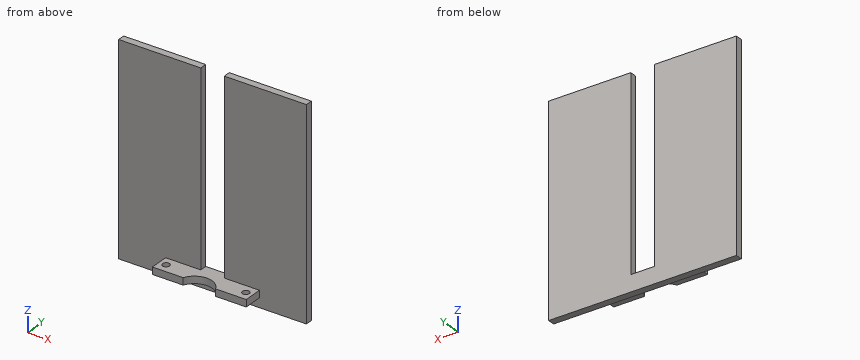
```python
from build123d import *

# Parameters (mm, degrees)
SKETCH2_R           = 1.5
BOSS_EXTRUDE1_DEPTH = 3
BOSS_EXTRUDE2_DEPTH = 3


with BuildPart() as part:
    # Sketch2 → Boss-Extrude1 (new body)
    with BuildSketch(Plane.XY):
        with BuildLine():
            Line((-20, 3), (-6.873863542, 3))
            ThreePointArc((-6.873863542, 3), (0, 7.5), (6.873863542, 3))
            Line((6.873863542, 3), (20, 3))
            Line((20, 3), (20, 11))
            Line((20, 11), (-20, 11))
            Line((-20, 11), (-20, 3))
        make_face()
        with Locations((-17, 7)):
            Circle(SKETCH2_R, mode=Mode.SUBTRACT)
        with Locations((17, 7)):
            Circle(SKETCH2_R, mode=Mode.SUBTRACT)
    extrude(amount=BOSS_EXTRUDE1_DEPTH)

    # Sketch3 → Boss-Extrude2 (add)
    with BuildSketch(Plane(origin=(0, 11, 0), x_dir=(1, 0, 0), z_dir=(0, 1, 0))):
        Polygon((-5, -84), (-40, -84), (-40, 0), (-40, 4), (40, 4), (40, 0), (40, -84), (5, -84), (5, -3), (-5, -3), align=None)
    extrude(amount=BOSS_EXTRUDE2_DEPTH)


solid = part.part
```
Geometry check sheet. Reference: the model listing, model coordinates, mm. Coordinates: 2 decimals unless noted, no trailing zeros. Order: outer loops, then holes, each group sorted by start corner. A loop starts at its lowest first (then second) coordinate and runs counter-clockwise, first axis right, second up.
Q1. Sectioned sample at B-B on x = 17. Record the cut outline in (y, z).
Reply:
outline: (3, 0) - (5.5, 0) - (5.5, 3) - (3, 3) - close; (8.5, 0) - (11, 0) - (11, -4) - (14, -4) - (14, 84) - (11, 84) - (11, 3) - (8.5, 3) - close
Q2. Thickness scan on probe 1 along Y at (x, z) = (-17, 1); probe 2 along Y at (x, z) = (-35.5, 76); probe 3 along Z at (x, y) = (19, 6.5). Record the ranges inside material, lowest first.
Reply:
probe 1: y = 3 to 5.5, 8.5 to 14
probe 2: y = 11 to 14
probe 3: z = 0 to 3
Q3. Sectioned sample at A-A on z = 28.5. Record the cut outline in (x, y).
Reply:
outline: (-40, 11) - (-5, 11) - (-5, 14) - (-40, 14) - close; (5, 11) - (40, 11) - (40, 14) - (5, 14) - close
Q4. Sectioned sample at D-D on x = 33. Record the cut outline in (y, z).
Reply:
outline: (11, -4) - (14, -4) - (14, 84) - (11, 84) - close
Q5. Sectioned sample at C-C on y = 10. Record the cut outline in (x, z).
Reply:
outline: (-20, 0) - (20, 0) - (20, 3) - (-20, 3) - close
Q6. Depth check by flat-ended pin: pin 1 Ø1 at (x, y) = (10, 4.5) entering from -Z; pin 2 Ø3.5 at (y, z) = (5, 1) entering from +X; pin 3 Ø4 at (x, y) = (-4, 8) entering from +Z. Enter the tip coordinate at first touch or a pass-through.
Reply:
pin 1: stops at z = 0
pin 2: stops at x = 20
pin 3: stops at z = 3
